```python
from build123d import *
from OCP.BRepFilletAPI import BRepFilletAPI_MakeFillet

# Parameters (mm, degrees)
END_CHAMFER_1_6X45_SIZE  = 1.6
SHOULDER_FILLETS_R2_R    = 2
KEYWAY_START             = 35
KEYWAY_1_DEPTH_7_5_DEPTH = 7.5
KEYWAY_START_2           = 45
KEYWAY_2_DEPTH_9_DEPTH   = 9
KEYWAY_EDGE_FILLETS_R1   = 0.3
KEYWAY_EDGE_FILLETS_R2   = 0.5


with BuildPart() as part:
    # Shaft Profile Sketch → Stepped Shaft Body (revolve)
    with BuildSketch(Plane(origin=(0, 0, 0), x_dir=(0, 0, -1), z_dir=(1, 0, 0)), mode=Mode.PRIVATE) as stepped_shaft_body_sk:
        Polygon((-224, 0), (-224, -35), (-84, -35), (-84, -40), (0, -40), (0, -45), (188, -45), (188, -40), (246, -40), (246, 0), align=None)
    revolve(stepped_shaft_body_sk.sketch.rotate(Axis((0, 0, 224), (0, 0, -1)), 270), axis=Axis((0, 0, 224), (0, 0, -1)))

    # End Chamfer 1.6x45
    end_chamfer_1_6x45_edges = [part.edges().sort_by_distance(p)[0] for p in [
        (-35, 0, 224),
        (-40, 0, -246),
    ]]
    chamfer(end_chamfer_1_6x45_edges, length=END_CHAMFER_1_6X45_SIZE)

    # Shoulder Fillets R2
    shoulder_fillets_r2_edges = [part.edges().sort_by_distance(p)[0] for p in [
        (-40, 0, 0),
        (-35, 0, 84),
        (-40, 0, -188),
    ]]
    fillet(shoulder_fillets_r2_edges, radius=SHOULDER_FILLETS_R2_R)

    # Keyway Slots Sketch → Keyway 1 Depth 7.5 (cut)
    with BuildSketch(Plane(origin=(0, 0, 0), x_dir=(0, 0, -1), z_dir=(1, 0, 0)).offset(KEYWAY_START)):
        with BuildLine():
            Line((-209, 10), (-134, 10))
            ThreePointArc((-134, 10), (-124, 0), (-134, -10))
            Line((-134, -10), (-209, -10))
            ThreePointArc((-209, -10), (-219, 0), (-209, 10))
        make_face()
    extrude(amount=-KEYWAY_1_DEPTH_7_5_DEPTH, mode=Mode.SUBTRACT)

    # Sketch2_3 → Keyway 2 Depth 9 (cut)
    with BuildSketch(Plane(origin=(0, 0, 0), x_dir=(0, 0, -1), z_dir=(1, 0, 0)).offset(KEYWAY_START_2)):
        with BuildLine():
            Line((75.5, 12.5), (150.5, 12.5))
            ThreePointArc((150.5, 12.5), (163, 0), (150.5, -12.5))
            Line((150.5, -12.5), (75.5, -12.5))
            ThreePointArc((75.5, -12.5), (63, 0), (75.5, 12.5))
        make_face()
    extrude(amount=-KEYWAY_2_DEPTH_9_DEPTH, mode=Mode.SUBTRACT)

    # Keyway Edge Fillets: one fillet with a radius per group of edges: ONE call of the kernel's fillet builder (fillet() takes one radius for all edges)
    keyway_edge_fillets_edges_1 = [part.edges().sort_by_distance(p)[0] for p in [
        (27.5, 0, 219),
        (27.5, 0, 124),
        (27.5, -10, 171.5),
        (27.5, 10, 171.5),
    ]]
    keyway_edge_fillets_edges_2 = [part.edges().sort_by_distance(p)[0] for p in [
        (36, 0, -163),
        (36, -12.5, -113),
        (36, 0, -63),
        (36, 12.5, -113),
    ]]
    keyway_edge_fillets = BRepFilletAPI_MakeFillet(part.part.solid().wrapped)
    for e in keyway_edge_fillets_edges_1:
        keyway_edge_fillets.Add(KEYWAY_EDGE_FILLETS_R1, e.wrapped)
    for e in keyway_edge_fillets_edges_2:
        keyway_edge_fillets.Add(KEYWAY_EDGE_FILLETS_R2, e.wrapped)
    add(Compound.cast(keyway_edge_fillets.Shape()), mode=Mode.REPLACE)


solid = part.part
```
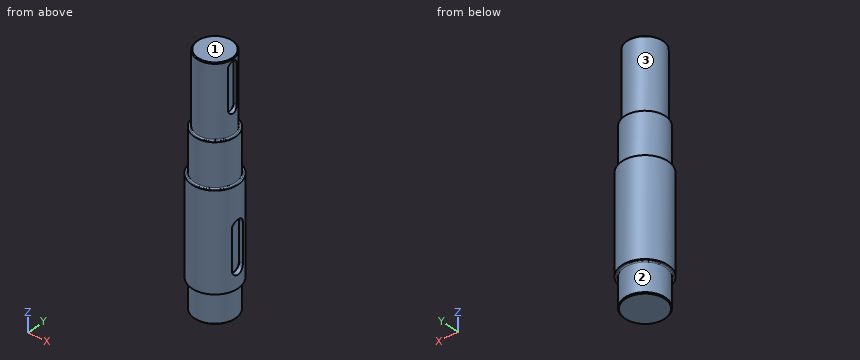
Verification items for the finished model (mm, model axes). Face numbers are marked on the shaded views. A direction names the side the tool comes from. Round coordinates to 2 decimals unless told otherwise and drop trailing zeros. Order: outer loops, then holes, each group sorted by start corner. A loop starts at its lowest first (then second) coordinate and runs counter-clockwise, first axis right, second up. Notation, with made-up numbers: (-25.75, -24) - (17.25, -24) arc R16 ccw to (17.25, -1) - close; hole circle Ø4 at (46, 63.5). An arc over 180 degrees is marked (long way). Use CSV: the item, a comma, the result in double quotes.
(1) Access from +Z, -Z, +X, -X, +Y, -Y to the whole of each face (thin tool, end or side, straight path). Record for the marked faces 1, 2 and 3.
Entries:
face 1,"+Z, +X, -X, +Y, -Y"
face 2,"-Z"
face 3,"+Z"
(2) Section check C-C on z = -174. Record the boundary of the cut face in (x, y).
Entries:
outline,"circle Ø90 at (0, 0)"
(3) Gauge pin test, flat ends, axial feed: pin 1 Ø5 at (x, z) = (-1.5, -194.5) entering from -Y; pin 2 Ø4.5 at (x, z) = (32, 189) entering from -Y; pin 3 Ø12 at (y, z) = (-2, -118.5) entering from +X. Record the tip position at first contact, or that the pin passes through.
Entries:
pin 1,"y = -40"
pin 2,"y = -18.44"
pin 3,"x = 36"
(4) Thickness scan on probe 1 along Z at (x, y) = (31, -12.5); probe 2 along X at (y, z) = (7, 0.5); probe 3 along Z at (x, y) = (39.5, -13). Record the ranges inside material, lowest first. Write a range as from..to.
Entries:
probe 1,"-246..223.97"
probe 2,"-40.07..40.07"
probe 3,"-188.04..0.04"
(5) Section check B-B on z = 94. Record the boundary of the cut face in (x, y), and give its area (3 significant figures).
Entries:
outline,"circle Ø70 at (0, 0)"
area,"3,850 mm^2"
(6) Section check A-A on x = 0. Record the boundary of the cut face in (y, z).
Entries:
outline,"(-45, -188) - (-42, -188) arc R2 cw to (-40, -190) - (-40, -244.4) - (-38.4, -246) - (38.4, -246) - (40, -244.4) - (40, -190) arc R2 cw to (42, -188) - (45, -188) - (45, 0) - (42, 0) arc R2 cw to (40, 2) - (40, 84) - (37, 84) arc R2 cw to (35, 86) - (35, 222.4) - (33.4, 224) - (-33.4, 224) - (-35, 222.4) - (-35, 86) arc R2 cw to (-37, 84) - (-40, 84) - (-40, 2) arc R2 cw to (-42, 0) - (-45, 0) - close"
